Geometry check sheet. Reference: the model listing, model coordinates, mm. A direction names the side the tool comes from. Round coordinates to 2 decimals unless told otherwise and drop trailing zeros. Write each loop counter-clockwise with the first axis right and the second up, starting at its lowest first coordinate (ties: lowest second). Pieces come first, ordered by that corner, then holes. Notation, with made-up numbers: (82.5, 13) -> (103.5, 13) arc R26 cw to (103.5, 45) -> close; hole circle Ø4 at (-31.5, 15). An arc over 180 degrees is marked (long way). Use a Markdown table: item, result.
```python
from build123d import *

# Parameters (mm, degrees)
SKETCH_1_W              = 193.5
SKETCH_1_H              = 80
EXTRUDE_1_DEPTH         = 7.5
HOLE_WIZARD_25_0_25_1_D = 25
HOLE_WIZARD_15_0_15_1_D = 15
HOLE_WIZARD_M8_1_D      = 6.8
HOLE_WIZARD_M8_1_DEPTH  = 19.75
HOLE_WIZARD_M8_1_TIP    = 2.042926105
HOLE_WIZARD_M8_2_D      = 6.8
HOLE_WIZARD_M8_2_DEPTH  = 19.75
HOLE_WIZARD_M8_2_TIP    = 2.042926105
SKETCH_11_R             = 56
CUT_EXTRUDE_1_DEPTH     = 10
CHAMFER_1_SIZE          = 2


with BuildPart() as part:
    # 草图1 → 凸台-拉伸1 (new, symmetric)
    with BuildSketch(Plane.XY):
        Rectangle(SKETCH_1_W, SKETCH_1_H)
    extrude(amount=EXTRUDE_1_DEPTH, both=True)

    # Ø25.0 (25) 直径孔1 (through all)
    with Locations(Plane.XY.offset(7.5)):
        with Locations((56.75, 0)):
            Hole(HOLE_WIZARD_25_0_25_1_D / 2)

    # Ø15.0 (15) 直径孔1 (through all)
    with Locations(Plane.XY.offset(7.5)):
        with Locations((-14.25, 30), (-14.25, -30)):
            Hole(HOLE_WIZARD_15_0_15_1_D / 2)

    # M8 螺纹孔1
    with Locations(Plane(origin=(96.75, 0, 0), x_dir=(0, 0, -1), z_dir=(1, 0, 0))):
        with Locations((0, 30), (0, -30)):
            Hole(HOLE_WIZARD_M8_1_D / 2, depth=HOLE_WIZARD_M8_1_DEPTH)
            with Locations((0, 0, -(HOLE_WIZARD_M8_1_DEPTH + HOLE_WIZARD_M8_1_TIP / 2))):  # 118° drill point
                Cone(0, HOLE_WIZARD_M8_1_D / 2, HOLE_WIZARD_M8_1_TIP, mode=Mode.SUBTRACT)

    # M8 螺纹孔2
    with Locations(Plane.ZY.offset(96.75)):
        with Locations((0, 30), (0, -30)):
            Hole(HOLE_WIZARD_M8_2_D / 2, depth=HOLE_WIZARD_M8_2_DEPTH)
            with Locations((0, 0, -(HOLE_WIZARD_M8_2_DEPTH + HOLE_WIZARD_M8_2_TIP / 2))):  # 118° drill point
                Cone(0, HOLE_WIZARD_M8_2_D / 2, HOLE_WIZARD_M8_2_TIP, mode=Mode.SUBTRACT)

    # 草图11 → 切除-拉伸1 (cut)
    with BuildSketch(Plane.ZY.offset(96.75)):
        with Locations((-52.5, 0)):
            Circle(SKETCH_11_R)
    extrude(amount=-CUT_EXTRUDE_1_DEPTH, mode=Mode.SUBTRACT)

    # 倒角1
    chamfer_1_edges = [part.edges().sort_by_distance(p)[0] for p in [
        (96.75, -40, 0),
        (-96.75, -40, 0),
        (-96.75, 40, 0),
        (96.75, 40, 0),
    ]]
    chamfer(chamfer_1_edges, length=CHAMFER_1_SIZE)


solid = part.part
```
(1) Section check D-D on x = 80.5. Record the cut outline in (y, z).
A:
| item | result |
|---|---|
| outline | (-40, -7.5) -> (40, -7.5) -> (40, 7.5) -> (-40, 7.5) -> close; hole circle Ø6.8 at (-30, 0); hole circle Ø6.8 at (30, 0) |
(2) Access from +Z, -Z, +X, -X, +Y, -Y to the whole of each face (thin tool, end or side, straight path). Record for faces 1 (the face through (86.74, 26.68, -0.74)), 2 (the face through (-86.74, 26.68, 0.74)), 3 (the face through (-91.82, -0.5, 3.498)).
A:
| item | result |
|---|---|
| face 1 | +X |
| face 2 | -X |
| face 3 | -Z, -X |
(3) Release check for a two-part mould opening along X. For faces 4 (the face through (-86.75, 0, -3)), 5 (the face through (69.238, 0.55, -0.105)), 6 (the face through (75.312, -30.576, 0.128)), 7 (the face through (-12.62, 22.68, -0.1)) record: +X half, -X half, draft (parallel to the pull), parting line (faces both ways), or undercut.
A:
| item | result |
|---|---|
| face 4 | -X half |
| face 5 | undercut |
| face 6 | +X half |
| face 7 | undercut |
(4) Thickness scan on line 1 (Y direction, x = -14.25, z = -1); line 2 (Y direction, x = 87, z = 0); line 3 (Z direction, x = 83, y = -30). Record the ranges inside material, lowest first.
A:
| item | result |
|---|---|
| line 1 | y = -40 to -37.5, -22.5 to 22.5, 37.5 to 40 |
| line 2 | y = -40 to -33.4, -26.6 to 26.6, 33.4 to 40 |
| line 3 | z = -7.5 to -3.4, 3.4 to 7.5 |
(5) Gauge pin test, flat ends, axial feed: pin 1 Ø5 at (y, z) = (-12.5, -5) entering from -X; pin 2 Ø4 at (y, z) = (-30, 0) entering from +X; pin 3 Ø9 at (y, z) = (30, 0) entering from +X; pin 4 Ø4 at (y, z) = (-30, 0) entering from -X. Record the tip position at first contact, or that the pin passes through.
A:
| item | result |
|---|---|
| pin 1 | stops at x = -86.75 |
| pin 2 | stops at x = 76.16 |
| pin 3 | stops at x = 96.75 |
| pin 4 | stops at x = -76.16 |
(6) Section check B-B on y = 0. Record the cut outline in (x, z), plus the area to 3 significant figures.
A:
| item | result |
|---|---|
| outline | (-96.75, 3.5) -> (-86.75, 3.5) -> (-86.75, -7.5) -> (44.25, -7.5) -> (44.25, 7.5) -> (-96.75, 7.5) -> close; (69.25, -7.5) -> (96.75, -7.5) -> (96.75, 7.5) -> (69.25, 7.5) -> close |
| area | 2,420 mm2 |
(7) Section check A-A on x = -14.25. Record the cut outline in (y, z), plus the area to 3 significant figures.
A:
| item | result |
|---|---|
| outline | (-40, -7.5) -> (-37.5, -7.5) -> (-37.5, 7.5) -> (-40, 7.5) -> close; (-22.5, -7.5) -> (22.5, -7.5) -> (22.5, 7.5) -> (-22.5, 7.5) -> close; (37.5, -7.5) -> (40, -7.5) -> (40, 7.5) -> (37.5, 7.5) -> close |
| area | 750 mm2 |
(8) Section check C-C on x = 56.75. Record the cut outline in (y, z).
A:
| item | result |
|---|---|
| outline | (-40, -7.5) -> (-12.5, -7.5) -> (-12.5, 7.5) -> (-40, 7.5) -> close; (12.5, -7.5) -> (40, -7.5) -> (40, 7.5) -> (12.5, 7.5) -> close |
